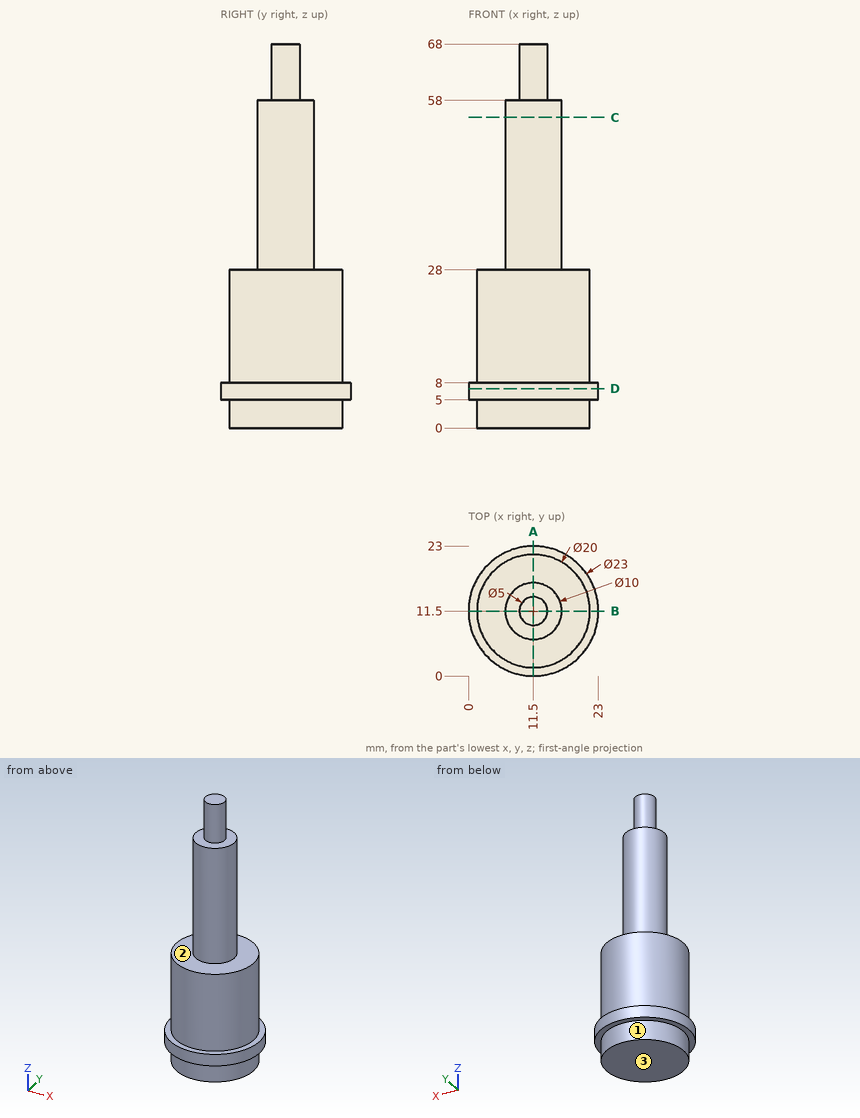
Check sheet for the drawn part. Datum: minimum x, y, z corner. Units: mm. A direction names the side the tool comes from. Round coordinates to 2 decimals unless told otherwise and drop trailing zeros. Order: outer loops, then holes, each group sorted by start corner. A loop starts at its lowest first (then second) coordinate and runs counter-clockwise, first axis right, second up. Notation, with made-up numbers: M 7.5,79.25 L 32.5,79.25 A18 ccw 32.5,90.25 Z; hole C -7.5,13.25 d3. An arc over 180 degrees is marked long. Write each question's results on one line, items separated by ' | '. Start each with the question number.
1. Cross-section at D-D on z = 7. Record the boundary of the cut face in (x, y), plus the area to 3 significant figures.
2. Cross-section at A-A on x = 11.5. Record the boundary of the cut face in (y, z).
3. Cross-section at C-C on z = 55. Record the boundary of the cut face in (x, y), plus the area to 3 significant figures.
4. Material ranges on L1, parallel to Z at x = 2.25, y = 8.75; L2, parallel to Z at x = 19, y = 20; L3, parallel to Y at x = 8.5, z = 29.5, recorded low to high. Write a range as from..to.
5. Go/stop test with flat-tipped pins: P1, Ø5, axis at x = 19, y = 15, coming from the -Z side; P2, Ø4, axis at x = 3.5, y = 4, coming from the +Z side; P3, Ø5, axis at x = 5.5, y = 15.5, coming from the +Z side; P4, Ø5, axis at y = 3.5, z = 40.5, coming from the +X side. Record where each tip stops, or that it passes through.
6. Set-up check for the marked faces 1, 2 and 3: record each of +Z, -Z, +X, -X, +Y, -Y from which the full face is reachable in a straight line by a thin tool's end or side.
Resolved:
1) outline: C 11.5,11.5 d23 | area: 415 mm2
2) outline: M 0,5 L 1.5,5 L 1.5,0 L 21.5,0 L 21.5,5 L 23,5 L 23,8 L 21.5,8 L 21.5,28 L 16.5,28 L 16.5,58 L 14,58 L 14,68 L 9,68 L 9,58 L 6.5,58 L 6.5,28 L 1.5,28 L 1.5,8 L 0,8 Z
3) outline: C 11.5,11.5 d10 | area: 78.5 mm2
4) L1: 0..28 | L2: 5..8 | L3: 7.5..15.5
5) P1: z = 0 | P2: z = 28 | P3: z = 58 | P4: through
6) face 1: -Z | face 2: +Z | face 3: -Z, +X, -X, +Y, -Y
